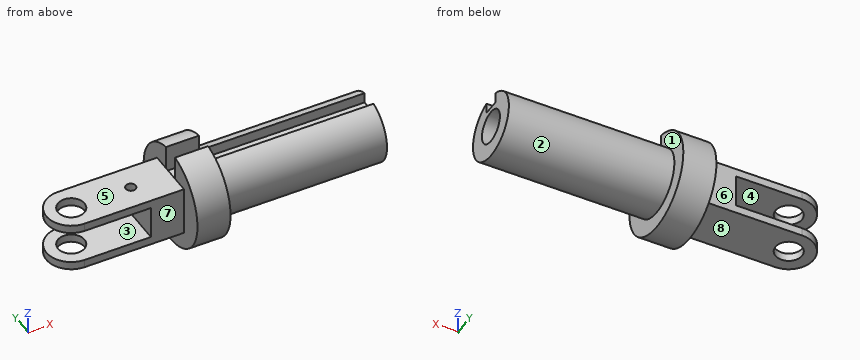
```python
from build123d import *

# Parameters (mm, degrees)
SKETCH2_R           = 0.4
BOSS_EXTRUDE1_DEPTH = 0.75
CUT_EXTRUDE1_DEPTH  = 0.5
SKETCH4_R           = 0.5
CUT_EXTRUDE2_DEPTH  = 6
CUT_EXTRUDE4_DEPTH  = 6
SKETCH6_R           = 0.15
CUT_EXTRUDE5_DEPTH  = 1


with BuildPart() as part:
    # Sketch1 → Revolve1 (revolve)
    with BuildSketch(Plane.XY, mode=Mode.PRIVATE) as revolve1_sk:
        Polygon((0, 0), (0, 1.5), (1, 1.5), (1, 1), (6, 1), (6, 0), align=None)
    revolve(revolve1_sk.sketch.rotate(Axis((0.124352332, 0, 0), (1, 0, 0)), 90), axis=Axis((0.124352332, 0, 0), (1, 0, 0)))

    # Sketch2 → Boss-Extrude1 (add, symmetric)
    with BuildSketch(Plane.XY):
        with BuildLine():
            Line((0, 0.75), (0, -0.75))
            Line((0, -0.75), (-3, -0.75))
            ThreePointArc((-3, -0.75), (-3.75, 0), (-3, 0.75))
            Line((-3, 0.75), (0, 0.75))
        make_face()
        with Locations((-3, 0)):
            Circle(SKETCH2_R, mode=Mode.SUBTRACT)
    extrude(amount=BOSS_EXTRUDE1_DEPTH, both=True)

    # Sketch3 → Cut-Extrude1 (cut, symmetric)
    with BuildSketch(Plane.XY):
        with BuildLine():
            Line((-1, 0.75), (-1, -0.75))
            Line((-1, -0.75), (-3, -0.75))
            ThreePointArc((-3, -0.75), (-3.75, 0), (-3, 0.75))
            Line((-3, 0.75), (-1, 0.75))
        make_face()
    extrude(amount=CUT_EXTRUDE1_DEPTH, both=True, mode=Mode.SUBTRACT)

    # Sketch4 → Cut-Extrude2 (cut)
    with BuildSketch(Plane(origin=(6, 0, 0), x_dir=(0, 0, -1), z_dir=(1, 0, 0))):
        Circle(SKETCH4_R)
    extrude(amount=-CUT_EXTRUDE2_DEPTH, mode=Mode.SUBTRACT)

    # Sketch5 → Cut-Extrude4 (cut)
    with BuildSketch(Plane(origin=(6, 0, 0), x_dir=(0, 0, -1), z_dir=(1, 0, 0))):
        with BuildLine():
            Line((-0.65, -0.25), (-0.65, 0.25))
            Line((-0.65, 0.25), (-0.968245837, 0.25))
            ThreePointArc((-0.968245837, 0.25), (-1, 0), (-0.968245837, -0.25))
            Line((-0.968245837, -0.25), (-0.65, -0.25))
        make_face()
        with BuildLine():
            ThreePointArc((-0.968245837, -0.25), (-1, 0), (-0.968245837, 0.25))
            Line((-0.968245837, 0.25), (-1.818815546, 0.25))
            Line((-1.818815546, 0.25), (-1.818815546, -0.25))
            Line((-1.818815546, -0.25), (-0.968245837, -0.25))
        make_face()
    extrude(amount=-CUT_EXTRUDE4_DEPTH, mode=Mode.SUBTRACT)

    # Sketch6 → Cut-Extrude5 (cut)
    with BuildSketch(Plane.XY.offset(0.75)):
        with Locations((-1.2, 0)):
            Circle(SKETCH6_R)
    extrude(amount=-CUT_EXTRUDE5_DEPTH, mode=Mode.SUBTRACT)


solid = part.part
```
Can you work these out from the model? Positions are in its coordinate system, mm. Face numbers are marked on the shaded views. A direction names the side the tool comes from. Coordinates: 2 decimals unless noted, no trailing zeros. Loops run counter-clockwise (first coordinate to the right, second up) from the corner with the lowest first, then second, coordinate; pieces in that order, holes last. Notation, with made-up numbers: (29, -38.75) -> (77, -38.75) arc R35 cw to (77, -1.75) -> close; hole circle Ø7 at (-2, -28). An arc over 180 degrees is marked (long way). Put each result on its own line as item: value. Start each with the question number.
Q1. I want a section at D-D (x = 4.5). Write out the boundary of the cut face in (y, z).
Q2. I want a section at B-B (y = 0). Count the separate pieces of the cut face and the enclosed holes in it, plus the area to 3 significant figures.
Q3. I want a section at A-A (x = -1.2). Write out the boundary of the cut face in (y, z).
Q4. For the marked faces 4, 5, 6, 7 and 8, which set-ups out of +Z, -Z, +X, -X, +Y, -Y let a thin tool reach every point of the face, with its end or its side?
Q5. I want a section at C-C (z = 0). Write out the boundary of the cut face in (x, y).
Q6. Thinking about a two-plate mould opening in Z: for the marked faces 1, 2 and 3, which applies, pulls with the +Z half, pulls with the -Z half, needs draft (parallel to the pull), parting line crosses it, or undercut?
Q7. If I drill on line 1 (Y direction, x = 4.65, z = 0); line 2 (Y direction, x = -3, z = -0.55); line 3 (Z direction, x = -3.25, y = -0.55), over which ranges is the centre line in solid material (lowest first)? Write a range as [from, to].
Q8. I'm going to push flat-ended pins straight in: P1, Ø1.2, axis at x = -2.5, y = 0, coming from the -Z side; P2, Ø0.8, axis at x = -1.5, z = 0, coming from the -Y side; P3, Ø1, axis at x = 2.5, y = 1, coming from the -Z side; P4, Ø0.8, axis at x = -2.5, y = 0, coming from the +Z side. Where does each tip first touch, or does it pass through?
Taken from the geometry:
1. outline: (-0.25, 0.65) -> (-0.25, 0.97) arc R1 ccw (long way) to (0.25, 0.97) -> (0.25, 0.65) -> close; hole circle Ø1 at (0, 0)
2. separate pieces: 4
2. enclosed holes: 0
2. area: 6.80 mm2
3. outline: (-0.75, -0.75) -> (0.75, -0.75) -> (0.75, -0.5) -> (-0.75, -0.5) -> close; (-0.75, 0.5) -> (-0.15, 0.5) -> (-0.15, 0.75) -> (-0.75, 0.75) -> close; (0.15, 0.5) -> (0.75, 0.5) -> (0.75, 0.75) -> (0.15, 0.75) -> close
4. face 4: -X, +Y, -Y
4. face 5: +Z, -X, +Y, -Y
4. face 6: +Z, -Z, -X, +Y
4. face 7: +Z, -Z, -X, -Y
4. face 8: -Z, -X, +Y, -Y
5. outline: (-1, -0.75) -> (0, -0.75) -> (0, -1.5) -> (1, -1.5) -> (1, -1) -> (6, -1) -> (6, -0.5) -> (0, -0.5) -> (0, 0.5) -> (6, 0.5) -> (6, 1) -> (1, 1) -> (1, 1.5) -> (0, 1.5) -> (0, 0.75) -> (-1, 0.75) -> close
6. face 1: needs draft
6. face 2: parting line crosses it
6. face 3: undercut
7. line 1: y = [-1, -0.5], [0.5, 1]
7. line 2: y = [-0.75, -0.4], [0.4, 0.75]
7. line 3: z = [-0.75, -0.5], [0.5, 0.75]
8. P1: stops at z = -0.75
8. P2: passes through
8. P3: stops at z = -0.87
8. P4: stops at z = 0.75
